Work out the finished part from the listing and answer in its coordinate system (mm). Face numbers are marked on the shaded views. A direction names the side the tool comes from. Coordinates: 2 decimals unless noted, no trailing zeros. Order: outer loops, then holes, each group sorted by start corner. A loop starts at its lowest first (then second) coordinate and runs counter-clockwise, first axis right, second up. Notation, with made-up numbers: M -11,33 L 41,33 A21 ccw 41,52 Z; hole C -33,45 d4. An arc over 180 degrees is marked long. Use a Markdown table: item, result.
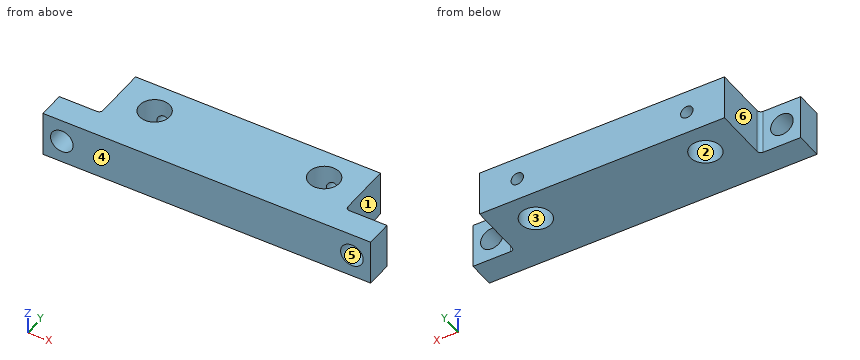
from build123d import *

# Parameters (mm, degrees)
SKETCH_1_R              = 4
EXTRUDE_1_DEPTH         = 6
HOLE_WIZARD_M4_1_REACH  = 71.828
HOLE_WIZARD_M4_1_BORE_R = 1.65
FILLET_1_R              = 1
CUT_EXTRUDE_1_REACH     = 48.403
SKETCH_3_R              = 3


with BuildPart() as part:
    # 草图1 → 凸台-拉伸1 (new, symmetric)
    with BuildSketch(Plane.XY):
        Polygon((0, 0), (-32.5, 0), (-32.5, -15), (-43.5, -15), (-43.5, -22), (43.5, -22), (43.5, -15), (32.5, -15), (32.5, 0), align=None)
        with Locations((-22.5, -8)):
            Circle(SKETCH_1_R, mode=Mode.SUBTRACT)
        with Locations((22.5, -8)):
            Circle(SKETCH_1_R, mode=Mode.SUBTRACT)
    extrude(amount=EXTRUDE_1_DEPTH, both=True)

    # M4 螺纹孔1 bore (on position points) → M4 螺纹孔1 (cut, up to next)
    with BuildSketch(Plane(origin=(-22.5, 0, 0), x_dir=(1, 0, 0), z_dir=(0, 1, 0)), mode=Mode.PRIVATE) as hole_wizard_m4_1_sk1:
        Circle(HOLE_WIZARD_M4_1_BORE_R)
    hole_wizard_m4_1_tool1 = extrude(hole_wizard_m4_1_sk1.sketch, amount=-HOLE_WIZARD_M4_1_REACH, mode=Mode.PRIVATE) & part.part
    hole_wizard_m4_1 = hole_wizard_m4_1_tool1.solids().sort_by_distance((-22.5, 0, 0))[0]
    add(hole_wizard_m4_1, mode=Mode.SUBTRACT)

    # 镜向1: M4 螺纹孔1 across plane
    add(hole_wizard_m4_1.mirror(Plane(origin=(0, 0, 0), x_dir=(0, 0, 1), z_dir=(1, 0, 0))), mode=Mode.SUBTRACT)

    # 圆角1
    fillet_1_edges = [part.edges().sort_by_distance(p)[0] for p in [
        (32.5, -15, 0),
        (-32.5, -15, 0),
    ]]
    fillet(fillet_1_edges, radius=FILLET_1_R)

    # 草图3 → 切除-拉伸1 (cut, up to next)
    with BuildSketch(Plane(origin=(0, -15, 0), x_dir=(1, 0, 0), z_dir=(0, 1, 0)), mode=Mode.PRIVATE) as cut_extrude_1_sk1:
        with Locations(Location((-38.5, 0, 0), (0, 0, 270))):
            Circle(SKETCH_3_R)
    cut_extrude_1_tool1 = extrude(cut_extrude_1_sk1.sketch, amount=-CUT_EXTRUDE_1_REACH, mode=Mode.PRIVATE) & part.part
    # 草图3 → 切除-拉伸1 (cut, up to next)
    with BuildSketch(Plane(origin=(0, -15, 0), x_dir=(1, 0, 0), z_dir=(0, 1, 0)), mode=Mode.PRIVATE) as cut_extrude_1_sk2:
        with Locations(Location((38.5, 0, 0), (0, 0, 270))):
            Circle(SKETCH_3_R)
    cut_extrude_1_tool2 = extrude(cut_extrude_1_sk2.sketch, amount=-CUT_EXTRUDE_1_REACH, mode=Mode.PRIVATE) & part.part
    add(cut_extrude_1_tool1.solids().sort_by_distance((-38.5, -15, 0))[0], mode=Mode.SUBTRACT)
    add(cut_extrude_1_tool2.solids().sort_by_distance((38.5, -15, 0))[0], mode=Mode.SUBTRACT)


solid = part.part
1. For the marked faces 5 and 6, determine the directions among +Z, -Z, +X, -X, +Y, -Y from which every point of the face is accessible in a straight line to the end or side of a thin tool.
Answers below:
| item | result |
|---|---|
| face 5 | +Y, -Y |
| face 6 | +Z, -Z, -X, +Y |
2. Flat-ended cylindrical pins translate along their axes: P1, Ø6.5, axis at x = -22.5, y = -8, coming from the -Z side; P2, Ø3, axis at x = 38.5, z = -2.5, coming from the +Y side; P3, Ø1.5, axis at y = -4, z = 4, coming from the -X side; P4, Ø1.5, axis at y = -3, z = -3.5, coming from the +X side. Find the tip coordinate at first contact, or state that the pin passes through.
Answers below:
| item | result |
|---|---|
| P1 | through |
| P2 | y = -15 |
| P3 | x = -32.5 |
| P4 | x = 32.5 |
3. For a pull along Y with two mould halves and no side action, classify the marked faces 1, 2, 3 and 4 as +Y half, -Y half, draft (parallel to the pull), parting line (faces both ways), or undercut.
Answers below:
| item | result |
|---|---|
| face 1 | draft |
| face 2 | undercut |
| face 3 | undercut |
| face 4 | -Y half |
4. Section B-B on y = -8 is taken. Determine the outline of the cut face in (x, z).
Answers below:
| item | result |
|---|---|
| outline | M -32.5,-6 L -26.5,-6 L -26.5,6 L -32.5,6 Z; M -18.5,-6 L 18.5,-6 L 18.5,6 L -18.5,6 Z; M 26.5,-6 L 32.5,-6 L 32.5,6 L 26.5,6 Z |
5. Section A-A on x = 38.5 is taken. Determine the outline of the cut face in (y, z).
Answers below:
| item | result |
|---|---|
| outline | M -22,-6 L -15,-6 L -15,-3 L -22,-3 Z; M -22,3 L -15,3 L -15,6 L -22,6 Z |
6. Find the intervals of material crossed by probe 1 along X at (y, z) = (-18.25, 0.25); probe 2 along Y at (x, z) = (-22.5, 3); probe 3 along X at (y, z) = (-4, 0.5), in increasing order.
Answers below:
| item | result |
|---|---|
| probe 1 | -43.5 to -41.49, -35.51 to 35.51, 41.49 to 43.5 |
| probe 2 | -22 to -12, -4 to 0 |
| probe 3 | -32.5 to -24.07, -20.93 to 20.93, 24.07 to 32.5 |
7. Section C-C on x = 22.5 is taken. Determine the outline of the cut face in (y, z), then the cut area to 3 significant figures.
Answers below:
| item | result |
|---|---|
| outline | M -22,-6 L -12,-6 L -12,6 L -22,6 Z; M -4,-6 L 0,-6 L 0,-1.65 L -4,-1.65 Z; M -4,1.65 L 0,1.65 L 0,6 L -4,6 Z |
| area | 155 mm² |
8. Section D-D on y = -3 is taken. Determine the outline of the cut face in (x, z), then the cut area to 3 significant figures.
Answers below:
| item | result |
|---|---|
| outline | M -32.5,-6 L 32.5,-6 L 32.5,6 L -32.5,6 Z; hole C -22.5,0 d3.3; hole C 22.5,0 d3.3 |
| area | 763 mm² |
